```python
from build123d import *

# Parameters (mm, degrees)
BOSS_EXTRUDE1_DEPTH = 100
SKETCH2_R           = 10
CUT_EXTRUDE1_DEPTH  = 100


with BuildPart() as part:
    # Sketch1 → Boss-Extrude1 (new body)
    with BuildSketch(Plane.XY):
        with BuildLine():
            Line((0, 0), (0, -120))
            Line((0, -120), (80, -120))
            Line((80, -120), (80, -108))
            Line((80, -108), (22, -108))
            ThreePointArc((22, -108), (14.928932188, -105.071067812), (12, -98))
            Line((12, -98), (12, 0))
            Line((12, 0), (0, 0))
        make_face()
    extrude(amount=BOSS_EXTRUDE1_DEPTH)

    # Sketch2 → Cut-Extrude1 (cut)
    with BuildSketch(Plane(origin=(0, -108, 0), x_dir=(1, 0, 0), z_dir=(0, 1, 0))):
        with Locations(Location((46, -50, 0), (0, 0, 270))):
            Circle(SKETCH2_R)
    extrude(amount=-CUT_EXTRUDE1_DEPTH, mode=Mode.SUBTRACT)


solid = part.part
```
Geometry check sheet. Reference: the model listing, model coordinates, mm. A direction names the side the tool comes from. Coordinates: 2 decimals unless noted, no trailing zeros. Write each loop counter-clockwise with the first axis right and the second up, starting at its lowest first coordinate (ties: lowest second). Pieces come first, ordered by that corner, then holes. Notation, with made-up numbers: (-38, -20.5) -> (-5, -20.5) arc R11 cw to (-5, -7.5) -> close; hole circle Ø3 at (2.5, 84). An arc over 180 degrees is marked (long way). Use CSV: the item, a comma, the result in double quotes. Start each with the question number.
Item 1: Cross-section at A-A, the plane x = 46. Record the cut outline in (y, z), plus the area to 3 significant figures.
Item 2: Depth check by flat-ended pin: pin 1 Ø8 at (y, z) = (-17.5, 49) entering from +X; pin 2 Ø1.5 at (x, z) = (32, 20.5) entering from +Y; pin 3 Ø1.5 at (y, z) = (-76.5, 41.5) entering from -X. Enter the tip coordinate at first touch or a pass-through.
Item 3: Cross-section at C-C, the plane z = 70. Record the cut outline in (x, y), plus the area to 3 significant figures.
Item 4: Cross-section at B-B, the plane z = 50. Record the cut outline in (x, y), plus the area to 3 significant figures.
Item 5: Cross-section at D-D, the plane x = 69.5. Record the cut outline in (y, z), plus the area to 3 significant figures.
Item 6: Thickness scan on line 1 (X direction, y = -110.25, z = 50); line 2 (Y direction, x = 26, z = 15.5); line 3 (X direction, y = -44.5, z = 74). Record the ranges inside material, lowest first.
Item 7: Set-up check for faces 4 (the flat face through (31, -120, 49)), 5 (the flat face through (12, -50, 49)): record each of +Z, -Z, +X, -X, +Y, -Y from which the full face is reachable in a straight line by a thin tool's end or side.
Item 8: Mould release check, pull along X, two halves, no side actions. Record for faces 1 (the flat face through (10, -82, 0)), 2 (the cylindrical face through (15.01, -105.15, 49.3)), 3 (the cylindrical face through (36.24, -113.92, 47.83)): released by +X, released by -X, zero draft, split by the parting line, or undercut.
Answers:
1,outline,"(-120, 0) -> (-108, 0) -> (-108, 40) -> (-120, 40) -> close; (-120, 60) -> (-108, 60) -> (-108, 100) -> (-120, 100) -> close"
1,area,"960 mm^2"
2,pin 1,"x = 12"
2,pin 2,"y = -108"
2,pin 3,"x = 0"
3,outline,"(0, -120) -> (80, -120) -> (80, -108) -> (22, -108) arc R10 cw to (12, -98) -> (12, 0) -> (0, 0) -> close"
3,area,"2,280 mm^2"
4,outline,"(0, -120) -> (36, -120) -> (36, -108) -> (22, -108) arc R10 cw to (12, -98) -> (12, 0) -> (0, 0) -> close; (56, -120) -> (80, -120) -> (80, -108) -> (56, -108) -> close"
4,area,"2,040 mm^2"
5,outline,"(-120, 0) -> (-108, 0) -> (-108, 100) -> (-120, 100) -> close"
5,area,"1,200 mm^2"
6,line 1,"0 to 36, 56 to 80"
6,line 2,"-120 to -108"
6,line 3,"0 to 12"
7,face 4,"+Z, -Z, +X, -X, -Y"
7,face 5,"+Z, -Z, +X, +Y"
8,face 1,"zero draft"
8,face 2,"released by +X"
8,face 3,"undercut"
